from build123d import *

# Parameters (mm, degrees)
BASE_PLATE_DEPTH       = 12
CLEVIS_BODY_PROFILE_W  = 14
CLEVIS_BODY_PROFILE_H  = 40
CLEVIS_BODY_DEPTH      = 60
CLEVIS_BODY_2_DEPTH    = 60
LUG_1_BOSS_SKETCH_R    = 30
LUG_1_BOSS_DEPTH       = 10
LUG_1_TRIM_SKETCH_W    = 60
LUG_1_TRIM_SKETCH_H    = 4
LUG_1_TRIM_DEPTH       = 40
LUG_2_BOSS_SKETCH_R    = 30
LUG_2_BOSS_DEPTH       = 10
LUG_2_TRIM_SKETCH_W    = 60
LUG_2_TRIM_SKETCH_H    = 4
LUG_2_TRIM_DEPTH       = 40
CLEVIS_WEB_SKETCH_W    = 60
CLEVIS_WEB_SKETCH_H    = 20
CLEVIS_WEB_DEPTH       = 10
PIN_HOLE_SKETCH_R      = 12.5
PIN_HOLE_25_DEPTH      = 40
COUNTERBORE_SKETCH_R   = 17.5
COUNTERBORE_35X6_DEPTH = 6
MOUNTING_HOLE_SKETCH_R = 10
MOUNTING_HOLE_20_DEPTH = 6


with BuildPart() as part:
    # Base Plate Profile → Base Plate (new body)
    with BuildSketch(Plane.XY):
        Polygon((-6, 0), (-6, -63), (6, -75), (42, -75), (54, -63), (54, 0), align=None)
    extrude(amount=BASE_PLATE_DEPTH)



with BuildPart() as body_2:
    # Clevis Body Profile → Clevis Body (new body)
    with BuildSketch(Plane.ZY.offset(6)):
        with Locations((19, 20)):
            Rectangle(CLEVIS_BODY_PROFILE_W, CLEVIS_BODY_PROFILE_H)
    extrude(amount=-CLEVIS_BODY_DEPTH)

    # Lug 2 Boss Sketch → Lug 2 Boss (add)
    with BuildSketch(Plane.XY.offset(26)):
        with Locations((24, 40)):
            Circle(LUG_2_BOSS_SKETCH_R)
    extrude(amount=-LUG_2_BOSS_DEPTH)

    # Lug 2 Trim Sketch → Lug 2 Trim (cut)
    with BuildSketch(Plane(origin=(0, 40, 0), x_dir=(1, 0, 0), z_dir=(0, 1, 0))):
        with Locations((24, -14)):
            Rectangle(LUG_2_TRIM_SKETCH_W, LUG_2_TRIM_SKETCH_H)
    extrude(amount=-LUG_2_TRIM_DEPTH, mode=Mode.SUBTRACT)


with BuildPart() as body_3:
    # Clevis Body Profile → Clevis Body 2 (new body)
    with BuildSketch(Plane.ZY.offset(6)):
        with Locations((-7, 20)):
            Rectangle(CLEVIS_BODY_PROFILE_W, CLEVIS_BODY_PROFILE_H)
    extrude(amount=-CLEVIS_BODY_2_DEPTH)

    # Lug 1 Boss Sketch → Lug 1 Boss (add)
    with BuildSketch(Plane(origin=(0, 0, -14), x_dir=(-1, 0, 0), z_dir=(0, 0, -1))):
        with Locations((-24, 40)):
            Circle(LUG_1_BOSS_SKETCH_R)
    extrude(amount=-LUG_1_BOSS_DEPTH)

    # Lug 1 Trim Sketch → Lug 1 Trim (cut)
    with BuildSketch(Plane(origin=(0, 40, 0), x_dir=(1, 0, 0), z_dir=(0, 1, 0))):
        with Locations((24, 2)):
            Rectangle(LUG_1_TRIM_SKETCH_W, LUG_1_TRIM_SKETCH_H)
    extrude(amount=-LUG_1_TRIM_DEPTH, mode=Mode.SUBTRACT)


with BuildPart() as part_1:
    add(part.part)

    add(body_2.part)  # Clevis Web merges body 2

    add(body_3.part)  # Clevis Web merges body 3
    # Clevis Web Sketch → Clevis Web (add)
    with BuildSketch(Plane(origin=(0, 0, 0), x_dir=(1, 0, 0), z_dir=(0, 1, 0))):
        with Locations((24, -6)):
            Rectangle(CLEVIS_WEB_SKETCH_W, CLEVIS_WEB_SKETCH_H)
    extrude(amount=CLEVIS_WEB_DEPTH)

    # Pin Hole Sketch → Pin Hole Ø25 (cut)
    with BuildSketch(Plane.XY.offset(26)):
        with Locations((24, 40)):
            Circle(PIN_HOLE_SKETCH_R)
    extrude(amount=-PIN_HOLE_25_DEPTH, mode=Mode.SUBTRACT)

    # Counterbore Sketch → Counterbore Ø35x6 (cut)
    with BuildSketch(Plane.XY.offset(12)):
        with Locations((24, -50)):
            Circle(COUNTERBORE_SKETCH_R)
    extrude(amount=-COUNTERBORE_35X6_DEPTH, mode=Mode.SUBTRACT)

    # Mounting Hole Sketch → Mounting Hole Ø20 (cut)
    with BuildSketch(Plane.XY.offset(6)):
        with Locations((24, -50)):
            Circle(MOUNTING_HOLE_SKETCH_R)
    extrude(amount=-MOUNTING_HOLE_20_DEPTH, mode=Mode.SUBTRACT)


solid = part_1.part
Check sheet for the modelled part. Datum: model origin and axes. Units: mm. A direction names the side the tool comes from. Give positions to 0.01 mm unless a question says otherwise; leave off trailing zeros. Write each loop counter-clockwise with the first axis right and the second up, starting at its lowest first coordinate (ties: lowest second). Pieces come first, ordered by that corner, then holes. Notation, with made-up numbers: (88.25, 82) -> (112.25, 82) arc R33 cw to (112.25, 112) -> close; hole circle Ø1 at (-3, -40). An arc over 180 degrees is marked (long way). One line per item, written item: value. Start each with the question number.
Item 1: Section check C-C on y = -50. Record the cut outline in (x, z), then the cut area to 3 significant figures.
Item 2: Section check A-A on x = 24. Record the cut outline in (y, z), then the cut area to 3 significant figures.
Item 3: Material ranges on probe 1 along Y at (x, z) = (24, 19); probe 2 along Y at (x, z) = (24, 3); probe 3 along Z at (x, y) = (43, 54), recorded low to high. Write a range as from..to.
Item 4: Tool access check on faces 1 (the flat face through (24, 10, 6)), 2 (the cylindrical face through (21.72, -32.65, 9.04)), 3 (the flat face through (24, -29, 12)). Record the directions out of +Z, -Z, +X, -X, +Y, -Y that give a thin tool (end or side, any length) a straight path to the whole face; none if there is none.
Item 5: Draft check along Y on faces 4 (the flat face through (24, 27, 26)), 5 (the flat face through (32, -58, 6)), 6 (the flat face through (24, 0, -7)), 7 (the cylindrical face through (24.66, 69.993, 21.07)). Enter one of: +Y half, -Y half, draft (parallel to the pull), parting line (faces both ways), or undercut.
Item 6: Gauge pin test, flat ends, axial feed: pin 1 (7 mm diameter, centred on x = 35, z = 22.5, fed in from -Y); pin 2 (2 mm diameter, centred on x = 5, z = 21.5, fed in from +Y); pin 3 (10 mm diameter, centred on x = 24, z = 6.5, fed in from +Y). Record the tip position at first contact, or that the pin passes through.
Item 7: Section check B-B on z = 9. Record the cut outline in (x, y), then the cut area to 3 significant figures.
Item 8: Section check D-D on y = -65. Record the cut outline in (x, z).
Results list:
1. outline: (-6, 0) -> (14, 0) -> (14, 6) -> (6.5, 6) -> (6.5, 12) -> (-6, 12) -> close; (34, 0) -> (54, 0) -> (54, 12) -> (41.5, 12) -> (41.5, 6) -> (34, 6) -> close
1. area: 390 mm²
2. outline: (-75, 0) -> (-60, 0) -> (-60, 6) -> (-67.5, 6) -> (-67.5, 12) -> (-75, 12) -> close; (-40, 0) -> (0, 0) -> (0, -14) -> (27.5, -14) -> (27.5, -4) -> (10, -4) -> (10, 16) -> (27.5, 16) -> (27.5, 26) -> (0, 26) -> (0, 12) -> (-32.5, 12) -> (-32.5, 6) -> (-40, 6) -> close; (52.5, -14) -> (70, -14) -> (70, -4) -> (52.5, -4) -> close; (52.5, 16) -> (70, 16) -> (70, 26) -> (52.5, 26) -> close
2. area: 1,670 mm²
3. probe 1: 0..27.5, 52.5..70
3. probe 2: -75..-60, -40..10
3. probe 3: -14..-4, 16..26
4. face 1: +X, -X, +Y
4. face 2: +Z
4. face 3: +Z, +X, -X, -Y
5. face 4: draft
5. face 5: undercut
5. face 6: -Y half
5. face 7: +Y half
6. pin 1: y = 0
6. pin 2: y = 64
6. pin 3: y = 10
7. outline: (-6, -63) -> (6, -75) -> (42, -75) -> (54, -63) -> (54, 10) -> (-6, 10) -> close; hole circle Ø35 at (24, -50)
7. area: 3,990 mm²
8. outline: (-4, 0) -> (52, 0) -> (52, 12) -> (33.01, 12) -> (33.01, 6) -> (14.99, 6) -> (14.99, 12) -> (-4, 12) -> close
